Read the model definition and answer for the solid it produces. Units are mm, in the model's axes. Face numbers are marked on the shaded views. Round coordinates to 2 decimals unless told otherwise and drop trailing zeros. Write each loop counter-clockwise with the first axis right and the second up, starting at its lowest first coordinate (ties: lowest second). Pieces come first, ordered by that corner, then holes. Notation, with made-up numbers: (-5.5, -14) - (49.5, -14) arc R14 cw to (49.5, -1) - close; hole circle Ø10 at (40, 56.25). An arc over 180 degrees is marked (long way). Use one line per item in the form item = value. Start each with the question number.
1) Consider line 1 along X through (y, z) = (24, 0); line 2 along X through (y, z) = (213, 0); line 3 along Z through (x, y) = (74, 14). Determine where each line is inside the solid, lowest interval first. Write a range as from..to.
2) For a pull along X with two mould halves and no side action, classify the marked faces 1 and 2 as released by +X, released by -X, zero draft, split by the parting line, or undercut.
3) The part is cut by section A-A, the plane y = 388. Give the vertices of the cut face in (x, z), plus the area to 3 significant figures.
4) Each of these flat-tipped pins is pushed along its axis until it touches: pin 1 (1 mm diameter, centred on x = 48.5, y = 293.5, fed in from -Z); pin 2 (1.5 mm diameter, centred on x = 92, y = 654, fed in from -Z); pin 3 (10 mm diameter, centred on x = 112.5, y = 443.5, fed in from -Z). Where does it stop, or does it pass through?
from build123d import *

# Parameters (mm, degrees)
SKETCH_2_R          = 70
CUT_EXTRUDE_1_DEPTH = 40
CUT_EXTRUDE_START   = -40
SKETCH_3_R          = 70
CUT_EXTRUDE_2_DEPTH = 40
SKETCH_4_R          = 69
CUT_EXTRUDE_3_DEPTH = 843
CHAMFER_1_SIZE      = 1


with BuildPart() as part:
    # 草图1 → 旋转1 (revolve)
    with BuildSketch(Plane.XY, mode=Mode.PRIVATE) as revolve_1_sk:
        Polygon((0, 0), (-0.5, 225), (-0.5, 625), (0, 850), (74.5, 850), (74.5, 0), align=None)
    revolve(revolve_1_sk.sketch.rotate(Axis((74.5, 850, 0), (0, -1, 0)), 270), axis=Axis((74.5, 850, 0), (0, -1, 0)))

    # 草图2 → 切除-拉伸1 (cut)
    with BuildSketch(Plane(origin=(0, 850, 0), x_dir=(1, 0, 0), z_dir=(0, 1, 0))):
        with Locations(Location((74.5, 0, 0), (0, 0, 270))):
            Circle(SKETCH_2_R)
    extrude(amount=-CUT_EXTRUDE_1_DEPTH, mode=Mode.SUBTRACT)

    # 草图3 → 切除-拉伸2 (cut)
    with BuildSketch(Plane.XZ.offset(CUT_EXTRUDE_START)):
        with Locations(Location((74.5, 0, 0), (0, 0, 90))):
            Circle(SKETCH_3_R)
    extrude(amount=CUT_EXTRUDE_2_DEPTH, mode=Mode.SUBTRACT)

    # 草图4 → 切除-拉伸3 (cut)
    with BuildSketch(Plane.XZ.offset(-40)):
        with Locations(Location((74.5, 0, 0), (0, 0, 270))):
            Circle(SKETCH_4_R)
    extrude(amount=-CUT_EXTRUDE_3_DEPTH, mode=Mode.SUBTRACT)

    # 倒角1
    chamfer_1_edges = [part.edges().sort_by_distance(p)[0] for p in [
        (74.5, 850, -70),
        (74.5, 0, -70),
    ]]
    chamfer(chamfer_1_edges, length=CHAMFER_1_SIZE)


solid = part.part
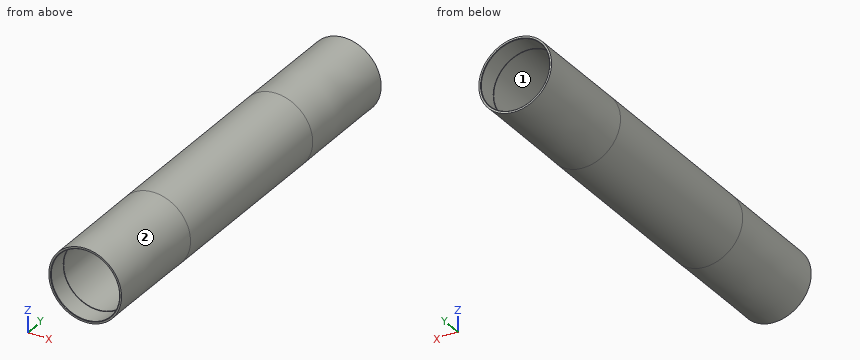
Geometry results:
q1.line_1 = -0.05..4.5, 144.5..149.05
q1.line_2 = -0.47..5.5, 143.5..149.47
q1.line_3 = -74.53..-70, 70..74.53
q2.face_1 = undercut
q2.face_2 = split by the parting line
q3.outline = circle Ø150 at (74.5, 0); hole circle Ø138 at (74.5, 0)
q3.area = 2,710 mm2
q4.pin_1 = -70.53
q4.pin_2 = -73.04
q4.pin_3 = -67.35
